Build history of the part. All positions in model axes, mm. A direction names the side the tool comes from. Coordinates: 2 decimals unless noted, no trailing zeros. Write each loop counter-clockwise with the first axis right and the second up, starting at its lowest first coordinate (ties: lowest second). Pieces come first, ordered by that corner, then holes.
```python
from build123d import *

# Parameters (mm, degrees)
EXTRUDE_1_DEPTH     = 95
CHAMFER_1_SIZE      = 5
CHAMFER_2_SIZE      = 2
CUT_EXTRUDE_1_REACH = 100.931


with BuildPart() as part:
    # 草图1 → 凸台-拉伸1 (new, symmetric)
    with BuildSketch(Plane.XY):
        Polygon((0, 0), (0, 22.5), (16, 22.5), (16, 17.5), (12, 17.5), (12, 0), align=None)
    extrude(amount=EXTRUDE_1_DEPTH, both=True)

    # 倒角1
    chamfer_1_edges = [part.edges().sort_by_distance(p)[0] for p in [
        (12, 8.75, 95),
        (12, 8.75, -95),
    ]]
    chamfer(chamfer_1_edges, length=CHAMFER_1_SIZE)

    # 倒角2
    chamfer_2_edges = [part.edges().sort_by_distance(p)[0] for p in [
        (16, 20, 95),
        (0, 11.25, 95),
        (0, 11.25, -95),
        (16, 20, -95),
    ]]
    chamfer(chamfer_2_edges, length=CHAMFER_2_SIZE)

    # 草图2 → 切除-拉伸1 (cut, up to next)
    with BuildSketch(Plane.XZ, mode=Mode.PRIVATE) as cut_extrude_1_sk1:
        with BuildLine():
            Line((4.5, 83), (7.5, 83))
            ThreePointArc((7.5, 83), (10, 80.5), (7.5, 78))
            Line((7.5, 78), (4.5, 78))
            ThreePointArc((4.5, 78), (2, 80.5), (4.5, 83))
        make_face()
    cut_extrude_1_tool1 = extrude(cut_extrude_1_sk1.sketch, amount=-CUT_EXTRUDE_1_REACH, mode=Mode.PRIVATE) & part.part
    # 草图2 → 切除-拉伸1 (cut, up to next)
    with BuildSketch(Plane.XZ, mode=Mode.PRIVATE) as cut_extrude_1_sk2:
        with BuildLine():
            Line((4.5, 2.5), (7.5, 2.5))
            ThreePointArc((7.5, 2.5), (10, 0), (7.5, -2.5))
            Line((7.5, -2.5), (4.5, -2.5))
            ThreePointArc((4.5, -2.5), (2, 0), (4.5, 2.5))
        make_face()
    cut_extrude_1_tool2 = extrude(cut_extrude_1_sk2.sketch, amount=-CUT_EXTRUDE_1_REACH, mode=Mode.PRIVATE) & part.part
    # 草图2 → 切除-拉伸1 (cut, up to next)
    with BuildSketch(Plane.XZ, mode=Mode.PRIVATE) as cut_extrude_1_sk3:
        with BuildLine():
            Line((4.5, -83), (7.5, -83))
            ThreePointArc((7.5, -83), (10, -80.5), (7.5, -78))
            Line((7.5, -78), (4.5, -78))
            ThreePointArc((4.5, -78), (2, -80.5), (4.5, -83))
        make_face()
    cut_extrude_1_tool3 = extrude(cut_extrude_1_sk3.sketch, amount=-CUT_EXTRUDE_1_REACH, mode=Mode.PRIVATE) & part.part
    add(cut_extrude_1_tool1.solids().sort_by_distance((6, 0, 80.5))[0], mode=Mode.SUBTRACT)
    add(cut_extrude_1_tool2.solids().sort_by_distance((6, 0, 0))[0], mode=Mode.SUBTRACT)
    add(cut_extrude_1_tool3.solids().sort_by_distance((6, 0, -80.5))[0], mode=Mode.SUBTRACT)


solid = part.part
```
1. Mould opens along Z. For faces 4 (the face through (5, 14, 95)), 5 (the face through (10, 0, 1)), 6 (the face through (10, 11, 0)) say: +Z half, -Z half, draft (parallel to the pull), parting line (faces both ways), or undercut.
Computed values:
face 4: +Z half
face 5: draft
face 6: undercut
2. Saw through at A-A on z = 80.5. List the corners of the cut face in (x, y).
Computed values:
outline: (0, 0) - (2, 0) - (2, 22.5) - (0, 22.5) - close; (10, 0) - (12, 0) - (12, 17.5) - (16, 17.5) - (16, 22.5) - (10, 22.5) - close
3. Saw through at C-C on z = -42.5. List the corners of the cut face in (x, y), plus the area to 3 significant figures.
Computed values:
outline: (0, 0) - (12, 0) - (12, 17.5) - (16, 17.5) - (16, 22.5) - (0, 22.5) - close
area: 290 mm2
4. 3-axis set-ups, long thin cutter, end or side, ignore diameter. For faces 1 (the face through (6, 11, 83)), 2 (the face through (12, 9, 1)), 3 (the face through (9, 9, -93)): which of +Z, -Z, +X, -X, +Y, -Y reach the whole face in a straight line?
Computed values:
face 1: +Y, -Y
face 2: +Z, -Z, +X, -Y
face 3: -Z, +X, -Y
5. Probe line 1 along Z through (x, y) = (4.5, 20.5); line 2 along Z through (x, y) = (7.5, 7); line 3 along Y through (x, z) = (14.75, 6). List the from-to ranges inside material, lowest first.
Computed values:
line 1: z = -95 to -83, -78 to -2.5, 2.5 to 78, 83 to 95
line 2: z = -94.5 to -83, -78 to -2.5, 2.5 to 78, 83 to 94.5
line 3: y = 17.5 to 22.5
6. Saw through at B-B on y = 5.75. List the corners of the cut face in (x, z).
Computed values:
outline: (0, -93) - (2, -95) - (7, -95) - (12, -90) - (12, 90) - (7, 95) - (2, 95) - (0, 93) - close; hole (4.5, -83) - (7.5, -83) arc R2.5 ccw to (7.5, -78) - (4.5, -78) arc R2.5 ccw to start; hole (4.5, -2.5) - (7.5, -2.5) arc R2.5 ccw to (7.5, 2.5) - (4.5, 2.5) arc R2.5 ccw to start; hole (4.5, 78) - (7.5, 78) arc R2.5 ccw to (7.5, 83) - (4.5, 83) arc R2.5 ccw to start
7. Flat gauge pins, fed straight in: pin 1 (1.5 mm diameter, centred on x = 10.5, y = 11, fed in from -Z); pin 2 (10 mm diameter, centred on y = 2.5, z = -7.5, fed in from +X); pin 3 (4 mm diameter, centred on x = 10.5, y = 12.5, fed in from +Z). Where does each tip first touch, or does it go through?
Computed values:
pin 1: stops at z = -92.25
pin 2: stops at x = 12
pin 3: stops at z = 93.5
